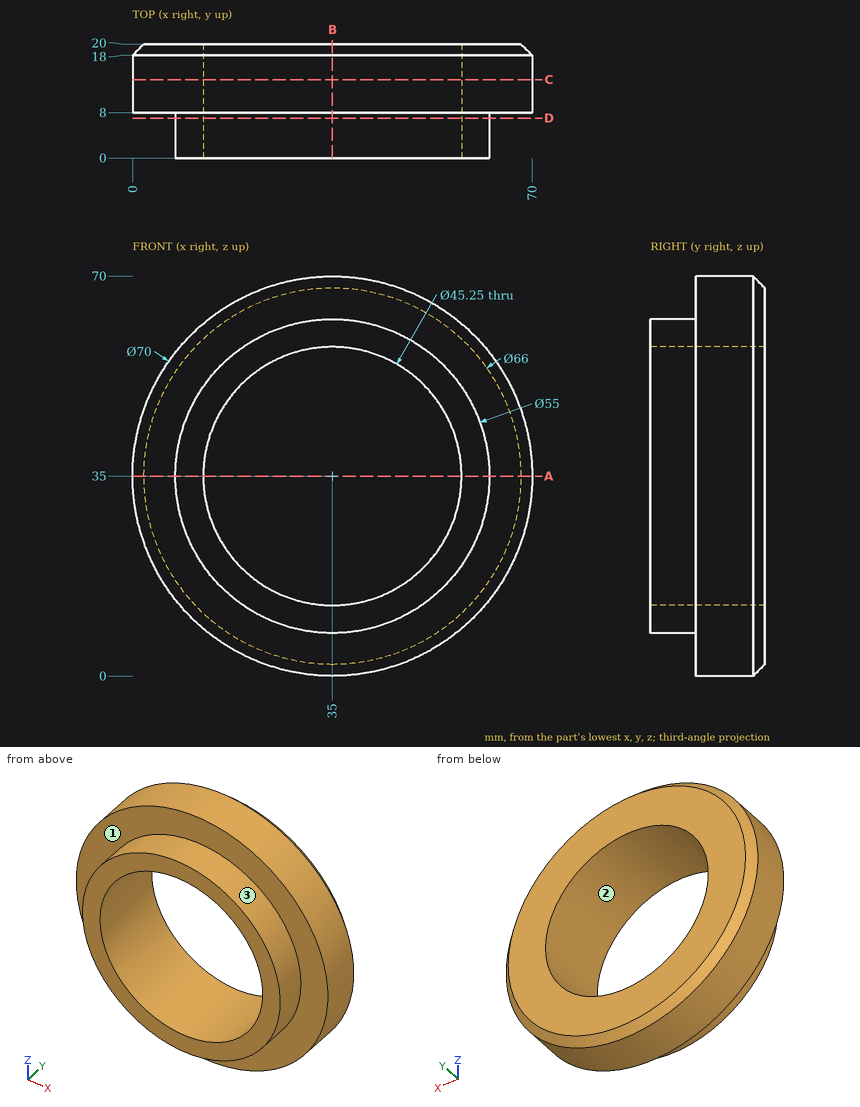
Here's the drawing with two shaded views (mm, measured from the low corner). I have some questions. Coordinates: 2 decimals unless noted, no trailing zeros. Loops run counter-clockwise (first coordinate to the right, second up) from the corner with the lowest first, then second, coordinate; pieces in that order, holes last. Notation, with made-up numbers: (51.5, 27) -> (78.5, 27) arc R10 ccw to (78.5, 45) -> close; hole circle Ø6 at (81, -36). An arc over 180 degrees is marked (long way). Put each result on its own line as item: value. Start each with the question number.
Q1. Thinking about a two-plate mould opening in Z: for the marked faces 1, 2 and 3, which applies, pulls with the +Z half, pulls with the -Z half, needs draft (parallel to the pull), parting line crosses it, or undercut?
Q2. I want a section at C-C (y = 13.75). Write out the boundary of the cut face in (x, z) (3 decimals).
Q3. I want a section at D-D (y = 7). Write out the boundary of the cut face in (x, z) (3 decimals).
Q4. I want a section at B-B (x = 35). Write out the boundary of the cut face in (y, z) (3 decimals), plus the area to 3 significant figures.
Q5. If I drill on line 1 (Y direction, x = 60.5, z = 23); line 2 (Z direction, x = 18.5, y = 18.5); line 3 (X direction, y = 12, z = 25.5), over which ranges is the centre line in solid material (lowest first)? Write a range as [from, to].
Q6. I'm going to push flat-ended pins straight in: P1, Ø2, axis at y = 16, z = 34.5, coming from the -X side; P2, Ø6, axis at y = 4.5, z = 33, coming from the +X side; P3, Ø1, axis at x = 63, y = 16.5, coming from the +Z side. Where does each tip first touch, or does it pass through?
Q7. I want a section at A-A (z = 35). Write out the boundary of the cut face in (x, y) (3 decimals).
Taken from the geometry:
1. face 1: needs draft
1. face 2: undercut
1. face 3: parting line crosses it
2. outline: circle Ø70 at (35, 35); hole circle Ø45.25 at (35, 35)
3. outline: circle Ø55 at (35, 35); hole circle Ø45.25 at (35, 35)
4. outline: (0, 7.5) -> (8, 7.5) -> (8, 0) -> (18, 0) -> (20, 2) -> (20, 12.375) -> (0, 12.375) -> close; (0, 57.625) -> (20, 57.625) -> (20, 68) -> (18, 70) -> (8, 70) -> (8, 62.5) -> (0, 62.5) -> close
4. area: 371 mm2
5. line 1: y = [8, 20]
5. line 2: z = [4.7, 19.52], [50.48, 65.3]
5. line 3: x = [1.31, 14.47], [55.53, 68.69]
6. P1: stops at x = 0
6. P2: stops at x = 62.5
6. P3: stops at z = 56.65
7. outline: (0, 8) -> (7.5, 8) -> (7.5, 0) -> (12.375, 0) -> (12.375, 20) -> (2, 20) -> (0, 18) -> close; (57.625, 0) -> (62.5, 0) -> (62.5, 8) -> (70, 8) -> (70, 18) -> (68, 20) -> (57.625, 20) -> close
